```python
from build123d import *

# Parameters (mm, degrees)
SKETCH1_R           = 20
BOSS_EXTRUDE1_DEPTH = 28
SKETCH2_R           = 27
BOSS_EXTRUDE2_DEPTH = 10
SKETCH3_R           = 15
BOSS_EXTRUDE3_DEPTH = 88
CHAMFER1_SIZE       = 1
CHAMFER2_SIZE       = 2
CUT_EXTRUDE2_START  = -11
CUT_EXTRUDE2_DEPTH  = 11


with BuildPart() as part:
    # Sketch1 → Boss-Extrude1 (new body)
    with BuildSketch(Plane(origin=(0, 0, 0), x_dir=(1, 0, 0), z_dir=(0, 1, 0))):
        with Locations(Location((0, 0, 0), (0, 0, 270))):
            Circle(SKETCH1_R)
    extrude(amount=BOSS_EXTRUDE1_DEPTH)

    # Sketch2 → Boss-Extrude2 (add)
    with BuildSketch(Plane(origin=(0, 28, 0), x_dir=(1, 0, 0), z_dir=(0, 1, 0))):
        with Locations(Location((0, 0, 0), (0, 0, 270))):
            Circle(SKETCH2_R)
    extrude(amount=BOSS_EXTRUDE2_DEPTH)

    # Sketch3 → Boss-Extrude3 (add)
    with BuildSketch(Plane.XZ):
        with Locations(Location((0, 0, 0), (0, 0, 90))):
            Circle(SKETCH3_R)
    extrude(amount=BOSS_EXTRUDE3_DEPTH)

    # Chamfer1
    chamfer1_edges = [part.edges().sort_by_distance(p)[0] for p in [
        (0, -88, -15),
        (0, 28, -27),
        (0, 38, -27),
    ]]
    chamfer(chamfer1_edges, length=CHAMFER1_SIZE)

    # Chamfer2
    chamfer2_edges = [part.edges().sort_by_distance(p)[0] for p in [
        (0, 0, -20),
    ]]
    chamfer(chamfer2_edges, length=CHAMFER2_SIZE)

    # Sketch5 → Cut-Extrude2 (cut)
    with BuildSketch(Plane.XY.offset(CUT_EXTRUDE2_START)):
        with BuildLine():
            Line((-2.4, -100.6), (2.4, -100.6))
            Line((2.4, -100.6), (2.4, -75.4))
            ThreePointArc((2.4, -75.4), (0, -73), (-2.4, -75.4))
            Line((-2.4, -75.4), (-2.4, -100.6))
        make_face()
    extrude(amount=-CUT_EXTRUDE2_DEPTH, mode=Mode.SUBTRACT)


solid = part.part
```
The listing builds one solid part. Answer for the finished solid, in the listing's coordinates (mm). A direction names the side the tool comes from. Coordinates: 2 decimals unless noted, no trailing zeros. Write each loop counter-clockwise with the first axis right and the second up, starting at its lowest first coordinate (ties: lowest second). Pieces come first, ordered by that corner, then holes. Notation, with made-up numbers: (78.5, 55) -> (93.5, 55) arc R23 cw to (93.5, 81) -> close; hole circle Ø9 at (0.5, -9.75). An arc over 180 degrees is marked (long way). Write each question's results on one line, items separated by ' | '. Start each with the question number.
1) A cutting plane is placed at C-C (y = -38). Determine the outline of the cut face in (x, z).
2) A cutting plane is placed at A-A (x = 0). Determine the outline of the cut face in (y, z), then the cut area to 3 significant figures.
3) Straight lines are drawn through the part: probe 1 along Y at (x, z) = (24.5, -3.5); probe 2 along Y at (x, z) = (16, -2); probe 3 along X at (y, z) = (-42.5, -4). For each, find the intervals that lie inside material, in ascending order.
4) A cutting plane is placed at B-B (z = 0). Determine the outline of the cut face in (x, y), then the cut area to 3 significant figures.
5) For a pull along X with two mould halves and no side action, classify faces 4 (the cylindrical face through (0, -73, -13)), 5 (the flat face through (2.4, -82, -13)), 6 (the cylindrical face through (5.745, -42.891, 13.856)), 7 (the flat face through (0, -88, 0)) as +X half, -X half, draft (parallel to the pull), parting line (faces both ways), or undercut.
6) Flat-ended cylindrical pins translate along their axes: pin 1 Ø3 at (x, z) = (17.5, -4.5) entering from -Y; pin 2 Ø4 at (y, z) = (-79.5, -13) entering from -X; pin 3 Ø10 at (x, y) = (13.5, -65.5) entering from -Z. Find the tip coordinate at first contact, or state that the pin passes through.
7) A tool of negligible diameter and unlimited length cuts with its end or side. For faces 1 (the flat face through (0, -80, -11)), 2 (the cylindrical face through (-26.36, 32.94, -5.85)), 3 (the flat face through (-15.3, 28, 13.4)), from which of +Z, -Z, +X, -X, +Y, -Y can it reach the whole face along a straight path? Write none if from no direction.
8) A cutting plane is placed at D-D (y = 11.5). Determine the outline of the cut face in (x, z), then the cut area to 3 significant figures.
Values follow:
1) outline: circle Ø30 at (0, 0)
2) outline: (-88, -11) -> (-73, -11) -> (-73, -15) -> (0, -15) -> (0, -18) -> (2, -20) -> (28, -20) -> (28, -26) -> (29, -27) -> (37, -27) -> (38, -26) -> (38, 26) -> (37, 27) -> (29, 27) -> (28, 26) -> (28, 20) -> (2, 20) -> (0, 18) -> (0, 15) -> (-87, 15) -> (-88, 14) -> close | area: 4,230 mm²
3) probe 1: 28 to 38 | probe 2: 0 to 38 | probe 3: -14.46 to 14.46
4) outline: (-27, 29) -> (-26, 28) -> (-20, 28) -> (-20, 2) -> (-18, 0) -> (-15, 0) -> (-15, -87) -> (-14, -88) -> (14, -88) -> (15, -87) -> (15, 0) -> (18, 0) -> (20, 2) -> (20, 28) -> (26, 28) -> (27, 29) -> (27, 37) -> (26, 38) -> (-26, 38) -> (-27, 37) -> close | area: 4,290 mm²
5) face 4: undercut | face 5: undercut | face 6: parting line | face 7: draft
6) pin 1: y = 0 | pin 2: x = -10.2 | pin 3: z = -12.36
7) face 1: -Z, -Y | face 2: +Y, -Y | face 3: -Y
8) outline: circle Ø40 at (0, 0) | area: 1,260 mm²
